```python
from build123d import *

# Parameters (mm, degrees)
SKETCH_1_W                = 200
SKETCH_1_H                = 120
EXTRUDE_1_DEPTH           = 20
HOLE_WIZARD_1_D           = 11
HOLE_WIZARD_1_CBORE_D     = 18
HOLE_WIZARD_1_CBORE_DEPTH = 11
HOLE_WIZARD_M14_1_D       = 12
CHAMFER_1_SIZE            = 5


with BuildPart() as part:
    # 草图1 → 凸台-拉伸1 (new body)
    with BuildSketch(Plane(origin=(0, 0, 0), x_dir=(0, 0, -1), z_dir=(1, 0, 0))):
        Rectangle(SKETCH_1_W, SKETCH_1_H)
    extrude(amount=EXTRUDE_1_DEPTH)

    # 打孔尺寸(%根据)内六角圆柱头螺钉的类型1 (through all)
    with Locations(Plane(origin=(20, 0, 0), x_dir=(0, 0, -1), z_dir=(1, 0, 0))):
        with Locations((30, 30), (-30, -30)):
            CounterBoreHole(HOLE_WIZARD_1_D / 2, HOLE_WIZARD_1_CBORE_D / 2, HOLE_WIZARD_1_CBORE_DEPTH)

    # M14 螺纹孔1 (through all)
    with Locations(Plane(origin=(20, 0, 0), x_dir=(0, 0, -1), z_dir=(1, 0, 0))):
        with Locations((-75, 0), (75, 0)):
            Hole(HOLE_WIZARD_M14_1_D / 2)

    # 倒角1
    chamfer_1_edges = [part.edges().sort_by_distance(p)[0] for p in [
        (10, -60, -100),
        (10, -60, 100),
        (10, 60, 100),
        (10, 60, -100),
    ]]
    chamfer(chamfer_1_edges, length=CHAMFER_1_SIZE)


solid = part.part
```
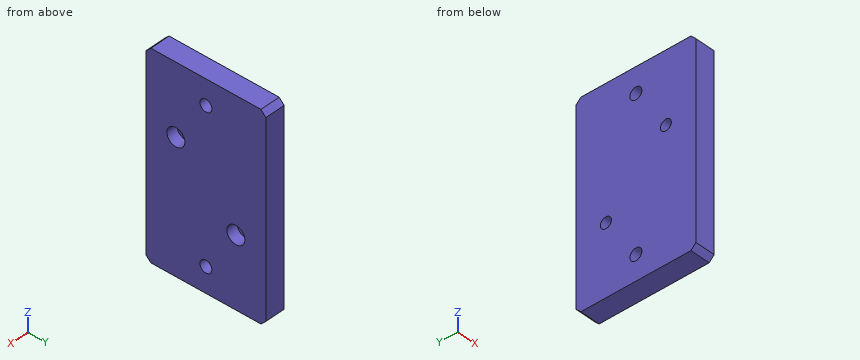
Input: part model. Units: mm. Frame: model coordinates. Give positions to 0.01 mm unless a question says otherwise; leave off trailing zeros. Order: outer loops, then holes, each group sorted by start corner. A loop starts at its lowest first (then second) coordinate and runs counter-clockwise, first axis right, second up.
1. Pin query (flat end, axial travel): pin 1 Ø6.5 at (y, z) = (30, -30) entering from -X; pin 2 Ø4 at (y, z) = (-29, -66) entering from -X; pin 3 Ø14.5 at (y, z) = (-30, 30) entering from +X. Return the tip coordinate at first contact, or that it passes through.
Computed:
pin 1: passes through
pin 2: stops at x = 0
pin 3: stops at x = 9
2. Cut plane C-C (z = 75). Return loops of the section in (x, y).
Computed:
outline: (0, -60) - (20, -60) - (20, -6) - (0, -6) - close; (0, 6) - (20, 6) - (20, 60) - (0, 60) - close
3. Cut plane A-A (x = 3.5). Return loops of the section in (y, z).
Computed:
outline: (-60, -95) - (-55, -100) - (55, -100) - (60, -95) - (60, 95) - (55, 100) - (-55, 100) - (-60, 95) - close; hole circle Ø11 at (-30, 30); hole circle Ø12 at (0, -75); hole circle Ø12 at (0, 75); hole circle Ø11 at (30, -30)
4. Cut plane B-B (y = 0). Return loops of the section in (x, z).
Computed:
outline: (0, -100) - (20, -100) - (20, -81) - (0, -81) - close; (0, -69) - (20, -69) - (20, 69) - (0, 69) - close; (0, 81) - (20, 81) - (20, 100) - (0, 100) - close
5. Cut plane D-D (y = -30). Return loops of the section in (x, z), and give its area (3 significant figures).
Computed:
outline: (0, -100) - (20, -100) - (20, 21) - (9, 21) - (9, 24.5) - (0, 24.5) - close; (0, 35.5) - (9, 35.5) - (9, 39) - (20, 39) - (20, 100) - (0, 100) - close
area: 3,700 mm2
6. Line query: probe 1 along Y at (x, z) = (9.5, 75); probe 2 along Y at (x, z) = (6, -30); probe 3 along X at (y, z) = (-36, 33). Output: solid intervals per line, ascending.
Computed:
probe 1: y = -60 to -6, 6 to 60
probe 2: y = -60 to 24.5, 35.5 to 60
probe 3: x = 0 to 9
